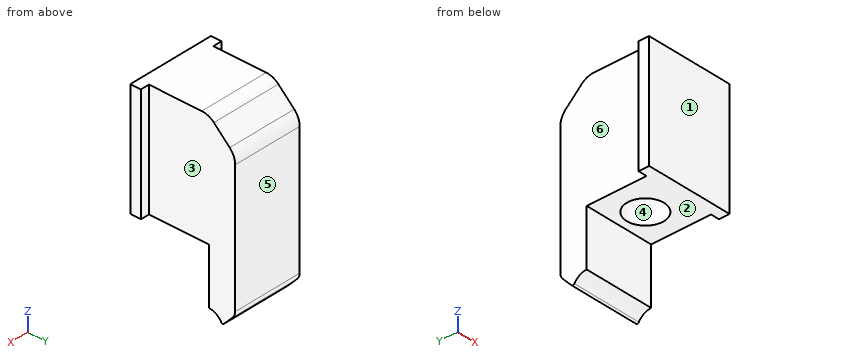
```python
from build123d import *

# Parameters (mm, degrees)
SKETCH1_W           = 50
SKETCH1_H           = 65
BOSS_EXTRUDE1_DEPTH = 6
SKETCH2_W           = 40
SKETCH2_H           = 65
BOSS_EXTRUDE2_DEPTH = 34
SKETCH3_R           = 10.5
CUT_EXTRUDE1_DEPTH  = 47
BOSS_EXTRUDE3_DEPTH = 20
FILLET1_R           = 10


with BuildPart() as part:
    # Sketch1 → Boss-Extrude1 (new body)
    with BuildSketch(Plane(origin=(0, 0, 0), x_dir=(1, 0, 0), z_dir=(0, 1, 0))):
        Rectangle(SKETCH1_W, SKETCH1_H)
    extrude(amount=BOSS_EXTRUDE1_DEPTH)

    # Sketch2 → Boss-Extrude2 (add)
    with BuildSketch(Plane(origin=(0, 6, 0), x_dir=(1, 0, 0), z_dir=(0, 1, 0))):
        Rectangle(SKETCH2_W, SKETCH2_H)
    extrude(amount=BOSS_EXTRUDE2_DEPTH)

    # Sketch3 → Cut-Extrude1 (cut)
    with BuildSketch(Plane(origin=(0, 0, -32.5), x_dir=(-1, 0, 0), z_dir=(0, 0, -1))):
        with Locations((0, 25)):
            Circle(SKETCH3_R)
    extrude(amount=-CUT_EXTRUDE1_DEPTH, mode=Mode.SUBTRACT)

    # Sketch4 → Boss-Extrude3 (add, symmetric)
    with BuildSketch(Plane(origin=(0, 0, 0), x_dir=(0, 0, -1), z_dir=(1, 0, 0))):
        with BuildLine():
            Line((-32.5, 40), (64.3, 40))
            ThreePointArc((64.3, 40), (65.360101389, 44.032598148), (68.266304348, 47.022522419))
            ThreePointArc((68.266304348, 47.022522419), (68.744948846, 47.778544361), (68.426967918, 48.614940117))
            Line((68.426967918, 48.614940117), (62.920069424, 53.680062627))
            ThreePointArc((62.920069424, 53.680062627), (61.351776951, 54.658342685), (59.535229833, 55))
            Line((59.535229833, 55), (28.36278807, 55))
            Line((28.36278807, 55), (-18.236030661, 55))
            Line((-18.236030661, 55), (-32.5, 40))
        make_face()
    extrude(amount=BOSS_EXTRUDE3_DEPTH, both=True)

    # Fillet1
    fillet1_edges = [part.edges().sort_by_distance(p)[0] for p in [
        (0, 40, 32.5),
        (0, 55, 18.236030661),
    ]]
    fillet(fillet1_edges, radius=FILLET1_R)


solid = part.part
```
The model under review builds one solid part; all positions refer to its coordinate system, in mm. Face numbers are marked on the shaded views. A direction names the side the tool comes from. Give positions to 0.01 mm unless a question says otherwise; leave off trailing zeros. Write each loop counter-clockwise with the first axis right and the second up, starting at its lowest first coordinate (ties: lowest second). Pieces come first, ordered by that corner, then holes. Notation, with made-up numbers: (83, -5.75) -> (127, -5.75) arc R20 cw to (127, 12.25) -> close; hole circle Ø5 at (46, 72). An arc over 180 degrees is marked (long way). Answer in a Markdown table with one row per item.
1) Add section C-C on x = 0. State the section outline as (y, z) points.
Worked answers:
| item | result |
|---|---|
| outline | (0, -32.5) -> (14.5, -32.5) -> (14.5, 14.5) -> (35.5, 14.5) -> (35.5, -32.5) -> (40, -32.5) -> (40, -64.3) arc R8.2 cw to (47.02, -68.27) arc R1 ccw to (48.61, -68.43) -> (53.68, -62.92) arc R5 ccw to (55, -59.54) -> (55, 13.95) arc R10 ccw to (51.89, 21.19) -> (42.9, 29.75) arc R10 ccw to (36, 32.5) -> (0, 32.5) -> close |
2) For L1, parallel to Y at x = 0, z = 1; L2, parallel to Y at x = -10.5, z = -46.5; L3, parallel to Z at x = 18.5, y = 21, list the stretches that pass through material, from the lowest coordinate up. Write a range as [from, to].
Worked answers:
| item | result |
|---|---|
| L1 | [0, 14.5], [35.5, 55] |
| L2 | [40, 55] |
| L3 | [-32.5, 32.5] |
3) Add section D-D on z = -38. State the section outline as (x, y) points.
Worked answers:
| item | result |
|---|---|
| outline | (-20, 40) -> (20, 40) -> (20, 55) -> (-20, 55) -> close |
4) Clearance check with flat-ended pins moving along their axes: P1, Ø10, axis at x = -7, y = 31, coming from the -Z side; P2, Ø4, axis at x = -13, y = 39.5, coming from the +Z side; P3, Ø2, axis at y = 35, z = 16, coming from the +X side. State where each tip first meets the part, or that it passes through.
Worked answers:
| item | result |
|---|---|
| P1 | z = -32.5 |
| P2 | z = 32.39 |
| P3 | x = 20 |
5) Tool access review of the marked faces 1 and 2: name each direction out of +Z, -Z, +X, -X, +Y, -Y from which nothing blocks a thin tool from reaching the whole face with its end or side.
Worked answers:
| item | result |
|---|---|
| face 1 | +Z, -Z, +X, -X, -Y |
| face 2 | -Z, +X, -X, -Y |
6) Add section A-A on z = -7. State the section outline as (x, y) points, plus the area to 3 significant figures.
Worked answers:
| item | result |
|---|---|
| outline | (-25, 0) -> (25, 0) -> (25, 6) -> (20, 6) -> (20, 55) -> (-20, 55) -> (-20, 6) -> (-25, 6) -> close; hole circle Ø21 at (0, 25) |
| area | 1,910 mm² |
7) Mouldability with a two-part tool opening along X and no side actions: class the marked faces 3, 4, 5 and 6 as +X half, -X half, draft (parallel to the pull), parting line (faces both ways), or undercut.
Worked answers:
| item | result |
|---|---|
| face 3 | +X half |
| face 4 | undercut |
| face 5 | draft |
| face 6 | -X half |
8) Add section B-B on y = 25. State the section outline as (x, z) points.
Worked answers:
| item | result |
|---|---|
| outline | (-20, -32.5) -> (-10.5, -32.5) -> (-10.5, 14.5) -> (10.5, 14.5) -> (10.5, -32.5) -> (20, -32.5) -> (20, 32.5) -> (-20, 32.5) -> close |
